Geometry check sheet. Reference: the model listing, model coordinates, mm. Face numbers are marked on the shaded views. Give positions to 0.01 mm unless a question says otherwise; leave off trailing zeros. Order: outer loops, then holes, each group sorted by start corner. A loop starts at its lowest first (then second) coordinate and runs counter-clockwise, first axis right, second up. Notation, with made-up numbers: M 43.5,34 L 89.5,34 A9 ccw 89.5,51 Z; hole C 81.5,11 d4. An arc over 180 degrees is marked long. Put each result on its own line as item: value. Start each with the question number.
Q1. Material ranges on L1, parallel to Y at x = 13, z = 0; L2, parallel to Z at x = 16.75, y = 5.25; L3, parallel to Y at x = 11.25, z = 6.5, recorded low to high.
Q2. Section check C-C on x = 15.75. Record the cut outline in (y, z).
Q3. Mould release check, pull along Y, two halves, no side actions. Record for the marked faces 1, 2, 3 and 4: +Y half, -Y half, draft (parallel to the pull), parting line (faces both ways), or undercut.
Q4. Go/stop test with flat-tipped pins: pin 1 (10 mm diameter, centred on y = 3, z = -1.5, fed in from +X); pin 2 (4 mm diameter, centred on x = 18, z = -8.5, fed in from +Y); pin 3 (3 mm diameter, centred on y = -9.5, z = -10, fed in from -X); pin 4 (9.5 mm diameter, centred on y = 0, z = 0, fed in from +X). Record where each tip stops, or that it passes through.
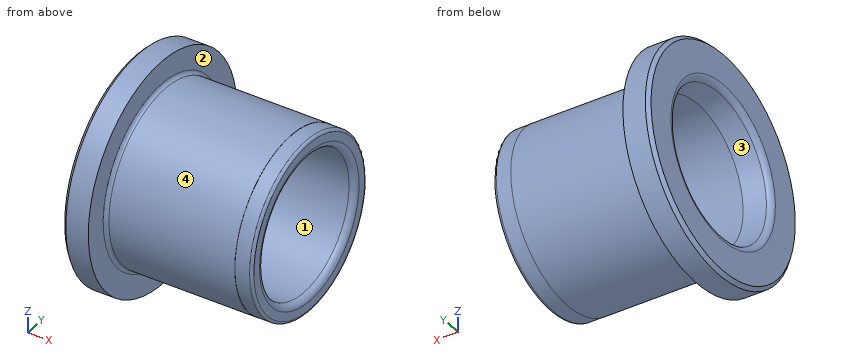
```python
from build123d import *


with BuildPart() as part:
    # Sketch1 → Revolve1 (revolve)
    with BuildSketch(Plane.XY, mode=Mode.PRIVATE) as revolve1_sk:
        with BuildLine():
            Line((0, 12.6), (0, 9.116350684))
            ThreePointArc((0, 9.116350684), (0.16376889, 8.666399357), (0.578446276, 8.426985257))
            Line((0.578446276, 8.426985257), (3, 8))
            Line((3, 8), (19.3, 8))
            ThreePointArc((19.3, 8), (19.794974747, 8.205025253), (20, 8.7))
            Line((20, 8.7), (20, 9.68))
            ThreePointArc((20, 9.68), (19.912132034, 9.892132034), (19.7, 9.98))
            Line((19.7, 9.98), (18, 9.98))
            Line((18, 9.98), (18, 10))
            Line((18, 10), (3.4, 10))
            ThreePointArc((3.4, 10), (3.117157288, 10.117157288), (3, 10.4))
            Line((3, 10.4), (3, 13))
            Line((3, 13), (0.4, 13))
            Line((0.4, 13), (0, 12.6))
        make_face()
    revolve(revolve1_sk.sketch.rotate(Axis((20, 0, 0), (-1, 0, 0)), 270), axis=Axis((20, 0, 0), (-1, 0, 0)))


solid = part.part
```
Results found:
1. L1: y = -10 to -8, 8 to 10
1. L2: z = -8.51 to -6.04, 6.04 to 8.51
1. L3: y = -7.6 to -4.66, 4.66 to 7.6
2. outline: C 0,0 d20; hole C 0,0 d16
3. face 1: undercut
3. face 2: draft
3. face 3: undercut
3. face 4: parting line
4. pin 1: stops at x = 19.91
4. pin 2: stops at y = 7.6
4. pin 3: stops at x = 0
4. pin 4: passes through
